```python
from build123d import *

# Parameters (mm, degrees)
SKETCH1_R                      = 10.5
SKETCH1_R_2                    = 6
BOSS_EXTRUDE1_DEPTH            = 28.5
BOSS_EXTRUDE2_START            = -6
SKETCH2_R                      = 21
SKETCH2_R_2                    = 6
BOSS_EXTRUDE2_DEPTH            = 6
F_7_5_7_5_DIAMETER_HOLE1_D     = 7.5
F_7_5_7_5_DIAMETER_HOLE1_DEPTH = 4.1
F_4_5_4_5_DIAMETER_HOLE1_D     = 4.5
CIRPATTERN1_COUNT              = 4
CUT_EXTRUDE1_START             = -6
SKETCH7_OUTSIDE_W              = 60.464
SKETCH7_OUTSIDE_H              = 60.464
CUT_EXTRUDE1_DEPTH             = 6


with BuildPart() as part:
    # Sketch1 → Boss-Extrude1 (new, symmetric)
    with BuildSketch(Plane(origin=(0, 0, 0), x_dir=(0, 0, -1), z_dir=(1, 0, 0))):
        with Locations(Location((0, 0, 0), (0, 0, 180))):
            Circle(SKETCH1_R)
        with Locations(Location((0, 0, 0), (0, 0, 180))):
            Circle(SKETCH1_R_2, mode=Mode.SUBTRACT)
    extrude(amount=BOSS_EXTRUDE1_DEPTH, both=True)

    # Sketch2 → Boss-Extrude2 (add)
    with BuildSketch(Plane(origin=(28.5, 0, 0), x_dir=(0, 0, -1), z_dir=(1, 0, 0)).offset(BOSS_EXTRUDE2_START)):
        Circle(SKETCH2_R)
        with Locations(Location((0, 0, 0), (0, 0, 180))):
            Circle(SKETCH2_R_2, mode=Mode.SUBTRACT)
    extrude(amount=BOSS_EXTRUDE2_DEPTH)

    # Ø7.5 (7.5) Diameter Hole1
    with Locations(Plane(origin=(28.5, 0, 0), x_dir=(0, 0, -1), z_dir=(1, 0, 0))):
        with Locations((0, 16)):
            f_7_5_7_5_diameter_hole1 = Hole(F_7_5_7_5_DIAMETER_HOLE1_D / 2, depth=F_7_5_7_5_DIAMETER_HOLE1_DEPTH)

    # Ø4.5 (4.5) Diameter Hole1 (through all)
    with Locations(Plane(origin=(24.4, 0, 0), x_dir=(0, 0, -1), z_dir=(1, 0, 0))):
        with Locations((0, 16)):
            f_4_5_4_5_diameter_hole1 = Hole(F_4_5_4_5_DIAMETER_HOLE1_D / 2)

    # CirPattern1: Ø7.5 (7.5) Diameter Hole1, Ø4.5 (4.5) Diameter Hole1 ×4 about axis
    cirpattern1_axis = Axis((0, 0, 0), (1, 0, 0))
    add([f_7_5_7_5_diameter_hole1.rotate(cirpattern1_axis, i * 360 / CIRPATTERN1_COUNT) for i in range(1, CIRPATTERN1_COUNT)], mode=Mode.SUBTRACT)
    add([f_4_5_4_5_diameter_hole1.rotate(cirpattern1_axis, i * 360 / CIRPATTERN1_COUNT) for i in range(1, CIRPATTERN1_COUNT)], mode=Mode.SUBTRACT)

    # Sketch7 outside → Cut-Extrude1 (cut)
    with BuildSketch(Plane(origin=(28.5, 0, 0), x_dir=(0, 0, -1), z_dir=(1, 0, 0)).offset(CUT_EXTRUDE1_START)):
        Rectangle(SKETCH7_OUTSIDE_W, SKETCH7_OUTSIDE_H)
        Polygon((0, 22.627416998), (-22.627416998, 0), (0, -22.627416998), (22.627416998, 0), align=None, mode=Mode.SUBTRACT)
    extrude(amount=CUT_EXTRUDE1_DEPTH, mode=Mode.SUBTRACT)


solid = part.part
```
Design review of the part built by this model. Coordinates are the model's own, in mm. A direction names the side the tool comes from. Round coordinates to 2 decimals unless told otherwise and drop trailing zeros. Write each loop counter-clockwise with the first axis right and the second up, starting at its lowest first coordinate (ties: lowest second). Pieces come first, ordered by that corner, then holes. Notation, with made-up numbers: (39, -14.75) -> (94, -14.75) arc R12 ccw to (94, -1.75) -> close; hole circle Ø11 at (-26, 29.25). An arc over 180 degrees is marked (long way). Answer in a Markdown table with one row per item.
Q1. Take a section at A-A, the plane y = 0. State the section outline as (x, z) points.
The answers:
| item | result |
|---|---|
| outline | (-28.5, -10.5) -> (22.5, -10.5) -> (22.5, -13.75) -> (24.4, -13.75) -> (24.4, -12.25) -> (28.5, -12.25) -> (28.5, -6) -> (-28.5, -6) -> close; (-28.5, 6) -> (28.5, 6) -> (28.5, 12.25) -> (24.4, 12.25) -> (24.4, 13.75) -> (22.5, 13.75) -> (22.5, 10.5) -> (-28.5, 10.5) -> close; (22.5, -21) -> (28.5, -21) -> (28.5, -19.75) -> (24.4, -19.75) -> (24.4, -18.25) -> (22.5, -18.25) -> close; (22.5, 18.25) -> (24.4, 18.25) -> (24.4, 19.75) -> (28.5, 19.75) -> (28.5, 21) -> (22.5, 21) -> close |
Q2. To check wall thickness, follow L1, parallel to Y at x = 8, z = 0; L2, parallel to Y at x = -23, z = 2.5; L3, parallel to X at y = 11.5, z = -0.5. State the ranges of each line that lie inside material, in increasing order. Write a range as [from, to].
The answers:
| item | result |
|---|---|
| L1 | [-10.5, -6], [6, 10.5] |
| L2 | [-10.2, -5.45], [5.45, 10.2] |
| L3 | [22.5, 28.5] |
Q3. Clearance check with flat-ended pins moving along their axes: pin 1 Ø8 at (y, z) = (-2, -17.5) entering from +X; pin 2 Ø10 at (y, z) = (16, 0) entering from -X; pin 3 Ø2 at (y, z) = (0, 17) entering from +X; pin 4 Ø4 at (x, z) = (16.5, 3.5) entering from -Y. State where each tip first meets the part, or that it passes through.
The answers:
| item | result |
|---|---|
| pin 1 | x = 28.5 |
| pin 2 | x = 22.5 |
| pin 3 | through |
| pin 4 | y = -10.39 |
Q4. For faces 5 (the face through (23.437, 0.488, 13.804)), 6 (the face through (26.42, 12.34, -0.81)), 7 (the face through (-2.6, -3.2, 10)), list the 3-axis set-ups (+Z, -Z, +X, -X, +Y, -Y) from which the entire face can be reached by the end or side of a thin tool; tool diameter is ignored.
The answers:
| item | result |
|---|---|
| face 5 | +X, -X |
| face 6 | +X |
| face 7 | -X |
Q5. Take a section at D-D, the plane z = -16. State the section outline as (x, y) points.
The answers:
| item | result |
|---|---|
| outline | (22.5, -6.63) -> (28.5, -6.63) -> (28.5, -3.75) -> (24.4, -3.75) -> (24.4, -2.25) -> (22.5, -2.25) -> close; (22.5, 2.25) -> (24.4, 2.25) -> (24.4, 3.75) -> (28.5, 3.75) -> (28.5, 6.63) -> (22.5, 6.63) -> close |
Q6. Draft analysis for pull direction Z (two halves, no side actions). For faces 1 (the face through (28.5, 6.3, -1.5)), 2 (the face through (24.4, -2, 14)), 3 (the face through (26.42, -12.34, 0.81)), 4 (the face through (25, 0, 21)), state which applies: +Z half, -Z half, draft (parallel to the pull), parting line (faces both ways), or undercut.
The answers:
| item | result |
|---|---|
| face 1 | draft |
| face 2 | undercut |
| face 3 | undercut |
| face 4 | +Z half |
Q7. Take a section at C-C, the plane y = -15. State the section outline as (x, z) points, then the cut area to 3 significant figures.
The answers:
| item | result |
|---|---|
| outline | (22.5, -7.63) -> (28.5, -7.63) -> (28.5, -3.61) -> (24.4, -3.61) -> (24.4, -2.02) -> (22.5, -2.02) -> close; (22.5, 2.02) -> (24.4, 2.02) -> (24.4, 3.61) -> (28.5, 3.61) -> (28.5, 7.63) -> (22.5, 7.63) -> close |
| area | 54.2 mm² |
